Model file for the job. Use its own axes, mm. A direction names the side the tool comes from. Coordinates: 2 decimals unless noted, no trailing zeros. Write each loop counter-clockwise with the first axis right and the second up, starting at its lowest first coordinate (ties: lowest second). Pieces come first, ordered by that corner, then holes. Notation, with made-up numbers: M 59,62.5 L 105,62.5 A14 cw 105,71.5 Z; hole C -14.5,-36.5 d5. An arc over 180 degrees is marked long. Answer in a Markdown table with one row per item. Add a question column.
```python
from build123d import *

# Parameters (mm, degrees)
EXTRUDE_387_DEPTH = 6.4
FILLET_1310_R     = 0.4


with BuildPart() as part:
    # 草图1 → Extrude 387 (new body)
    with BuildSketch(Plane(origin=(0, 0, 0), x_dir=(0, 0, -1), z_dir=(1, 0, 0))):
        Polygon((8, 4.618802154), (8, -4.618802154), (0, -9.237604307), (-8, -4.618802154), (-8, 4.618802154), (0, 9.237604307), align=None)
    extrude(amount=EXTRUDE_387_DEPTH)

    # 草图2 → 凸台-旋转1 (revolve)
    with BuildSketch(Plane.XY, mode=Mode.PRIVATE) as revolve_1_sk:
        Polygon((0, 0), (26.4, 0), (26.4, 3.701), (26.4, 5), (11.4, 5), (0, 5), align=None)
    revolve(revolve_1_sk.sketch.rotate(Axis((0, 0, 0), (1, 0, 0)), 90), axis=Axis((0, 0, 0), (1, 0, 0)))

    # 草图3 → 切除-旋转1 (revolve, cut)
    with BuildSketch(Plane.XY):
        Polygon((0, 8), (3.601282526, 14.237604307), (3.601282526, 19.237604307), (-10, 19.237604307), (-10, 8), align=None)
    revolve(axis=Axis((0, 0, 0), (1, 0, 0)), mode=Mode.SUBTRACT)

    # 草图4 → 切除-旋转3 (revolve, cut)
    with BuildSketch(Plane.XY, mode=Mode.PRIVATE) as cut_revolve_3_sk:
        Polygon((6.4, 7.315), (5.8, 7.661410162), (5.8, 9.237604307), (6.4, 9.237604307), align=None)
    revolve(cut_revolve_3_sk.sketch.rotate(Axis((0, 0, 0), (1, 0, 0)), 90), axis=Axis((0, 0, 0), (1, 0, 0)), mode=Mode.SUBTRACT)

    # Fillet 1310
    fillet_1310_edges = [part.edges().sort_by_distance(p)[0] for p in [
        (6.4, 0, -5),
    ]]
    fillet(fillet_1310_edges, radius=FILLET_1310_R)


solid = part.part
```
1) Slice it at B-B (x = 23). Give the cut face in (y, z).
2) Slice it at A-A (x = 2.5). Give the cut face in (y, z), then the cut area to 3 significant figures.
3) Flat gauge pins, fed straight in: pin 1 Ø6 at (x, z) = (11.5, 4) entering from +Y; pin 2 Ø3 at (y, z) = (5.5, -6) entering from +X; pin 3 Ø3 at (x, z) = (21, 1) entering from +Y. Where does each tip first touch, or does it go through?
4) Which spindle directions (+Z, -Z, +X, -X, +Y, -Y) get a long thin tool onto all of the face, cutting with end or side? Do faces 1 (the face through (26.4, 0, 0)), 2 (the face through (6.4, -5, -3)). Say none if no direction does.
5) Drill centre lines: probe 1 along X at (y, z) = (7, -0.25); probe 2 along Y at (x, z) = (20, -0.25); probe 3 along Y at (x, z) = (10.5, -3.5). Where is each one in solid material? Low to high.
Ans:
| question | item | result |
|---|---|---|
| 1 | outline | C 0,0 d10 |
| 2 | outline | M -9.24,0 L -4.62,-8 L 4.62,-8 L 9.24,0 L 4.62,8 L -4.62,8 Z |
| 2 | area | 222 mm2 |
| 3 | pin 1 | stops at y = 4.9 |
| 3 | pin 2 | stops at x = 6.4 |
| 3 | pin 3 | stops at y = 5 |
| 4 | face 1 | +Z, -Z, +X, +Y, -Y |
| 4 | face 2 | +X |
| 5 | probe 1 | x = 0 to 6.4 |
| 5 | probe 2 | y = -4.99 to 4.99 |
| 5 | probe 3 | y = -3.57 to 3.57 |
